Part model, mm, in its own coordinate system. A direction names the side the tool comes from. Give positions to 0.01 mm unless a question says otherwise; leave off trailing zeros. Order: outer loops, then holes, each group sorted by start corner. A loop starts at its lowest first (then second) coordinate and runs counter-clockwise, first axis right, second up. Notation, with made-up numbers: (60.25, -17.75) -> (119.25, -17.75) arc R17 cw to (119.25, -2.75) -> close; hole circle Ø7 at (82.25, -6.5). An arc over 180 degrees is marked (long way). Write item = value, one per line. Start each with the question number.
(1) Saw through at B-B, the plane z = 18. List the corners of the cut face in (x, y), then the cut area to 3 significant figures.
(2) Saw through at C-C, the plane x = 0. List the corners of the cut face in (y, z), then the cut area to 3 significant figures.
(3) Two-plate mould, pull along X, no slides. Class faces 6 (the cylindrical face through (12.1, 4.5, 6.5)), 7 (the flat face through (0, -9.5, 11)), 8 (the flat face through (-14, -6, 19.5)): pulls with the +X half, pulls with the -X half, needs draft (parallel to the pull), parting line crosses it, or undercut.
(4) Which spindle directions (+Z, -Z, +X, -X, +Y, -Y) get a long thin tool onto all of the face, cutting with end or side? Do faces 1 (the flat face through (0, 2, 8)), 2 (the flat face through (0, 0.5, 2)), 3 (the flat face through (0, -1, 0)), 4 (the flat face through (0, 6.6, 6)), 5 (the flat face through (-0.2, -9, 0.5)). Say none if no direction does.
(5) Flat gauge pins, fed straight in: pin 1 (1 mm diameter, centred on x = 0, z = 15, fed in from +Y); pin 2 (1 mm diameter, centred on x = 9.5, y = 7, fed in from +Z). Where does each tip first touch, or does it go through?
(6) Saw through at A-A, the plane x = 4. List the corners of the cut face in (y, z).
(7) Saw through at D-D, the plane z = 2.75. List the corners of the cut face in (x, y).
(8) Probe line 1 along Y through (x, z) = (4, 2.5); line 2 along Y through (x, z) = (0, 13.5); line 3 along X through (y, z) = (-6, 12.5). List the from-to ranges inside material, lowest first. Write a range as from..to.
from build123d import *

# Parameters (mm, degrees)
SKETCH_1_W                = 30
SKETCH_1_H                = 19
EXTRUDE_1_DEPTH           = 20.5
SKETCH_2_W                = 30
SKETCH_2_H                = 12
CUT_EXTRUDE_1_DEPTH       = 12.5
CUT_EXTRUDE_2_DEPTH       = 28.120103245
CUT_EXTRUDE_3_DEPTH       = 5
SKETCH_5_R                = 1.75
CUT_EXTRUDE_4_DEPTH       = 10
HOLE_WIZARD_M3_1_D        = 3.2
HOLE_WIZARD_M3_1_2_REACH  = 22.628
HOLE_WIZARD_M3_1_2_BORE_R = 1.25
CHAMFER_1_SIZE            = 2
CHAMFER_2_SIZE            = 1


with BuildPart() as part:
    # 草图1 → 凸台-拉伸1 (new body)
    with BuildSketch(Plane.XY):
        Rectangle(SKETCH_1_W, SKETCH_1_H)
    extrude(amount=EXTRUDE_1_DEPTH)

    # 草图2 → 切除-拉伸1 (cut)
    with BuildSketch(Plane.XY.offset(20.5)):
        with Locations((0, 3.5)):
            Rectangle(SKETCH_2_W, SKETCH_2_H)
    extrude(amount=-CUT_EXTRUDE_1_DEPTH, mode=Mode.SUBTRACT)

    # 草图3 → 切除-拉伸2 (cut, through all)
    with BuildSketch(Plane(origin=(0, 0, 0), x_dir=(-1, 0, 0), z_dir=(0, 0, -1))):
        with BuildLine():
            Line((10, 2.4), (-10, 2.4))
            ThreePointArc((-10, 2.4), (-12.1, 4.5), (-10, 6.6))
            Line((-10, 6.6), (10, 6.6))
            ThreePointArc((10, 6.6), (12.1, 4.5), (10, 2.4))
        make_face()
    extrude(amount=-CUT_EXTRUDE_2_DEPTH, mode=Mode.SUBTRACT)

    # 草图4 → 切除-拉伸3 (cut)
    with BuildSketch(Plane(origin=(0, 0, 0), x_dir=(-1, 0, 0), z_dir=(0, 0, -1))):
        with BuildLine():
            Line((10, 0.5), (-10, 0.5))
            ThreePointArc((-10, 0.5), (-14, 4.5), (-10, 8.5))
            Line((-10, 8.5), (10, 8.5))
            ThreePointArc((10, 8.5), (14, 4.5), (10, 0.5))
        make_face()
    extrude(amount=-CUT_EXTRUDE_3_DEPTH, mode=Mode.SUBTRACT)

    # 草图5 → 切除-拉伸4 (cut)
    with BuildSketch(Plane(origin=(0, 0, 0), x_dir=(-1, 0, 0), z_dir=(0, 0, -1))):
        with Locations((0, -6)):
            Circle(SKETCH_5_R)
    extrude(amount=-CUT_EXTRUDE_4_DEPTH, mode=Mode.SUBTRACT)

    # Hole Wizard M3 _1 (through all)
    with Locations(Plane(origin=(0, -9.5, 0), x_dir=(-1, 0, 0), z_dir=(0, -1, 0))):
        with Locations((0, -18)):
            Hole(HOLE_WIZARD_M3_1_D / 2)

    # Hole Wizard M3 _1 2 bore → Hole Wizard M3 _1 2 (cut, up to next)
    with BuildSketch(Plane(origin=(0, 0, 10), x_dir=(-1, 0, 0), z_dir=(0, 0, -1)), mode=Mode.PRIVATE) as hole_wizard_m3_1_2_sk1:
        with Locations((0, -6)):
            Circle(HOLE_WIZARD_M3_1_2_BORE_R)
    hole_wizard_m3_1_2_tool1 = extrude(hole_wizard_m3_1_2_sk1.sketch, amount=-HOLE_WIZARD_M3_1_2_REACH, mode=Mode.PRIVATE) & part.part
    add(hole_wizard_m3_1_2_tool1.solids().sort_by_distance((0, -6, 10))[0], mode=Mode.SUBTRACT)

    # 倒角1
    chamfer_1_edges = [part.edges().sort_by_distance(p)[0] for p in [
        (-15, -6, 20.5),
        (-15, 9.5, 4),
        (15, 9.5, 4),
        (15, -6, 20.5),
    ]]
    chamfer(chamfer_1_edges, length=CHAMFER_1_SIZE)

    # 倒角2
    chamfer_2_edges = [part.edges().sort_by_distance(p)[0] for p in [
        (0, -9.5, 0),
    ]]
    chamfer(chamfer_2_edges, length=CHAMFER_2_SIZE)


solid = part.part
Results list:
q1.outline = (-15, -9.5) -> (-1.6, -9.5) -> (-1.6, -2.5) -> (-15, -2.5) -> close; (1.6, -9.5) -> (15, -9.5) -> (15, -2.5) -> (1.6, -2.5) -> close
q1.area = 188 mm^2
q2.outline = (-9.5, 1) -> (-8.5, 0) -> (-7.75, 0) -> (-7.75, 10) -> (-7.25, 10) -> (-7.25, 16.4) -> (-9.5, 16.4) -> close; (-9.5, 19.6) -> (-2.5, 19.6) -> (-2.5, 20.5) -> (-9.5, 20.5) -> close; (-4.75, 10) -> (-4.25, 10) -> (-4.25, 0) -> (0.5, 0) -> (0.5, 5) -> (2.4, 5) -> (2.4, 8) -> (-2.5, 8) -> (-2.5, 16.4) -> (-4.75, 16.4) -> close; (6.6, 5) -> (8.5, 5) -> (8.5, 0) -> (9.5, 0) -> (9.5, 8) -> (6.6, 8) -> close
q2.area = 113 mm^2
q3.face_6 = undercut
q3.face_7 = needs draft
q3.face_8 = pulls with the -X half
q4.face_1 = +Z, +X, -X, +Y
q4.face_2 = -Z
q4.face_3 = -Z, +X, -X, +Y, -Y
q4.face_4 = +Z, -Z
q4.face_5 = -Z, +X, -X, -Y
q5.pin_1 = -2.5
q5.pin_2 = 8
q6.outline = (-9.5, 1) -> (-8.5, 0) -> (0.5, 0) -> (0.5, 5) -> (2.4, 5) -> (2.4, 8) -> (-2.5, 8) -> (-2.5, 20.5) -> (-9.5, 20.5) -> close; (6.6, 5) -> (8.5, 5) -> (8.5, 0) -> (9.5, 0) -> (9.5, 8) -> (6.6, 8) -> close
q7.outline = (-15, -9.5) -> (15, -9.5) -> (15, 7.5) -> (13, 9.5) -> (-13, 9.5) -> (-15, 7.5) -> close; hole (-10, 0.5) -> (10, 0.5) arc R4 ccw to (10, 8.5) -> (-10, 8.5) arc R4 ccw to start; hole circle Ø3.5 at (0, -6)
q8.line_1 = -9.5..0.5, 8.5..9.5
q8.line_2 = -9.5..-7.25, -4.75..-2.5
q8.line_3 = -15..-1.25, 1.25..15
